The model under review builds one solid part; all positions refer to its coordinate system, in mm. Face numbers are marked on the shaded views. A direction names the side the tool comes from. Give positions to 0.01 mm unless a question says otherwise; leave off trailing zeros. Write each loop counter-clockwise with the first axis right and the second up, starting at its lowest first coordinate (ties: lowest second). Pieces come first, ordered by that corner, then holes. Notation, with made-up numbers: (10.5, 46.25) -> (61.5, 46.25) arc R20 cw to (61.5, 77.25) -> close; hole circle Ø1 at (-4.5, -14.75). An arc over 180 degrees is marked (long way). Use CSV: the item, a comma, the result in double quotes.
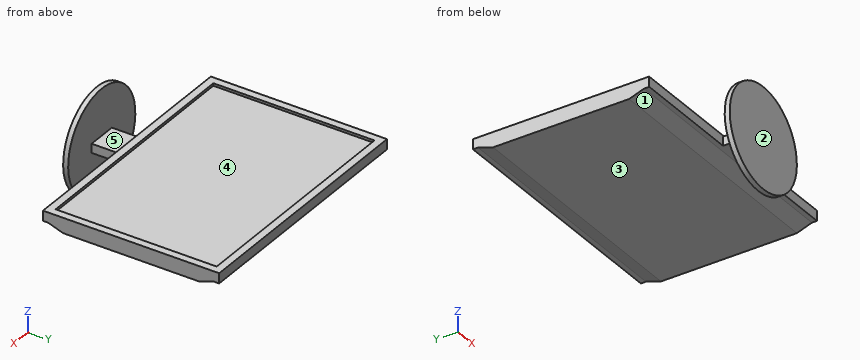
```python
from build123d import *

# Parameters (mm, degrees)
SKETCH1_W           = 500
SKETCH1_H           = 350
BOSS_EXTRUDE1_DEPTH = 20
BOSS_EXTRUDE2_DEPTH = 500
SKETCH3_W           = 470
SKETCH3_H           = 320
CUT_EXTRUDE1_DEPTH  = 5
SKETCH4_W           = 60
SKETCH4_H           = 18
BOSS_EXTRUDE3_DEPTH = 50
SKETCH5_R           = 100
BOSS_EXTRUDE4_DEPTH = 10


with BuildPart() as part:
    # Sketch1 → Boss-Extrude1 (new body)
    with BuildSketch(Plane.XY):
        with Locations((250, 175)):
            Rectangle(SKETCH1_W, SKETCH1_H)
    extrude(amount=BOSS_EXTRUDE1_DEPTH)

    # Sketch2 → Boss-Extrude2 (add)
    with BuildSketch(Plane(origin=(500, 0, 0), x_dir=(0, 0, -1), z_dir=(1, 0, 0))):
        Polygon((0, 340), (0, 10), (10, 40), (10, 310), align=None)
    extrude(amount=-BOSS_EXTRUDE2_DEPTH)

    # Sketch3 → Cut-Extrude1 (cut)
    with BuildSketch(Plane.XY.offset(20)):
        with Locations((250, 175)):
            Rectangle(SKETCH3_W, SKETCH3_H)
    extrude(amount=-CUT_EXTRUDE1_DEPTH, mode=Mode.SUBTRACT)

    # Sketch4 → Boss-Extrude3 (add)
    with BuildSketch(Plane.XZ):
        with Locations((250, 9)):
            Rectangle(SKETCH4_W, SKETCH4_H)
    extrude(amount=BOSS_EXTRUDE3_DEPTH)

    # Sketch5 → Boss-Extrude4 (add)
    with BuildSketch(Plane.XZ.offset(50)):
        with Locations(Location((250, 10, 0), (0, 0, 270))):
            Circle(SKETCH5_R)
    extrude(amount=BOSS_EXTRUDE4_DEPTH)


solid = part.part
```
Q1. Insertion check: pin 1 (8 mm diameter, centred on x = 215.5, y = 276, fed in from -Z); pin 2 (14.5 mm diameter, centred on y = -30, z = 10, fed in from +X); pin 3 (5 mm diameter, centred on x = 247.5, y = 343, fed in from -Z); pin 4 (4 mm diameter, centred on y = 112.5, z = 17, fed in from -X). Each pin has a flat end and moves straight along its axis. Give the tip position at first contact, or say it passes through.
Derived:
pin 1,"stops at z = -10"
pin 2,"stops at x = 280"
pin 3,"stops at z = 0"
pin 4,"stops at x = 0"
Q2. Consider section B-B (y = 316). Write out the cut boundary in (x, z).
Derived:
outline,"(0, -8) -> (500, -8) -> (500, 20) -> (485, 20) -> (485, 15) -> (15, 15) -> (15, 20) -> (0, 20) -> close"
Q3. The part is to be moulded in two halves that separate along Y. For the marked faces 1, 2 and 3, say which applies: pulls with the +Y half, pulls with the -Y half, needs draft (parallel to the pull), parting line crosses it, or undercut.
Derived:
face 1,"undercut"
face 2,"pulls with the -Y half"
face 3,"needs draft"
Q4. To check wall thickness, follow probe 1 along X at (y, z) = (68, 18); probe 2 along Z at (x, y) = (369, 160); probe 3 along Y at (x, z) = (267.5, -51). State the ranges of each line that lie inside material, in increasing order.
Derived:
probe 1,"x = 0 to 15, 485 to 500"
probe 2,"z = -10 to 15"
probe 3,"y = -60 to -50"
Q5. Consider section D-D (x = 250). Write out the cut boundary in (y, z), then the cut area to 3 significant figures.
Derived:
outline,"(-60, -90) -> (-50, -90) -> (-50, 0) -> (10, 0) -> (40, -10) -> (310, -10) -> (340, 0) -> (350, 0) -> (350, 20) -> (335, 20) -> (335, 15) -> (15, 15) -> (15, 20) -> (0, 20) -> (0, 18) -> (-50, 18) -> (-50, 110) -> (-60, 110) -> close"
area,"11,300 mm2"
Q6. Consider section A-A (x = 420.5). Write out the cut boundary in (y, z).
Derived:
outline,"(0, 0) -> (10, 0) -> (40, -10) -> (310, -10) -> (340, 0) -> (350, 0) -> (350, 20) -> (335, 20) -> (335, 15) -> (15, 15) -> (15, 20) -> (0, 20) -> close"
Q7. Consider section C-C (z = 8). Write out the cut boundary in (x, y), then the cut area to 3 significant figures.
Derived:
outline,"(0, 0) -> (220, 0) -> (220, -50) -> (150.02, -50) -> (150.02, -60) -> (349.98, -60) -> (349.98, -50) -> (280, -50) -> (280, 0) -> (500, 0) -> (500, 350) -> (0, 350) -> close"
area,"180,000 mm2"
Q8. Machinability: for the marked faces 4 and 5, which of the approach directions +Z, -Z, +X, -X, +Y, -Y give a long, thin tool a straight path to every point of the face, cutting with its end or side? Answer none if there is none.
Derived:
face 4,"+Z"
face 5,"+Z, +X, -X"
